The listing builds one solid part. Answer for the finished solid, in the listing's coordinates (mm). A direction names the side the tool comes from. Coordinates: 2 decimals unless noted, no trailing zeros. Order: outer loops, then holes, each group sorted by start corner. A loop starts at its lowest first (then second) coordinate and runs counter-clockwise, first axis right, second up. Notation, with made-up numbers: (65.25, -10) -> (88.25, -10) arc R22 ccw to (88.25, 24) -> close; hole circle Ø8 at (-3.75, 62.5). An arc over 180 degrees is marked (long way). Return JSON: item names as keys, results as strings.
```python
from build123d import *

# Parameters (mm, degrees)
SKETCH1_R                        = 9
BOSS_EXTRUDE1_DEPTH              = 40
M24_TAPPED_HOLE1_D               = 21
FILLET1_R                        = 10
SKETCH3_R                        = 9
SKETCH3_R_2                      = 9.680977079
BOSS_EXTRUDE2_DEPTH              = 25
M14_TAPPED_HOLE1_D               = 12
M14_TAPPED_HOLE1_DEPTH           = 40
M14_TAPPED_HOLE1_ON_FACE_2_D     = 12
M14_TAPPED_HOLE1_ON_FACE_2_DEPTH = 40


with BuildPart() as part:
    # Sketch1 → Boss-Extrude1 (new body)
    with BuildSketch(Plane.XY):
        Polygon((0, 215), (1520, 215), (1520, 120), (1420, 120), (1420, 0), (0, 0), align=None)
        with Locations((400, 166)):
            Circle(SKETCH1_R, mode=Mode.SUBTRACT)
        with Locations((280, 131)):
            Circle(SKETCH1_R, mode=Mode.SUBTRACT)
        with Locations((660, 131)):
            Circle(SKETCH1_R, mode=Mode.SUBTRACT)
        with Locations((1000, 166)):
            Circle(SKETCH1_R, mode=Mode.SUBTRACT)
    extrude(amount=BOSS_EXTRUDE1_DEPTH)

    # M24 Tapped Hole1 (through all)
    with Locations(Plane(origin=(780, 75, 40), x_dir=(1, 0, 0), z_dir=(0, 0, 1))):
        with Locations((0, 0), (-580, 0)):
            Hole(M24_TAPPED_HOLE1_D / 2)

    # Fillet1
    fillet1_edges = [part.edges().sort_by_distance(p)[0] for p in [
        (1520, 215, 20),
        (1520, 120, 20),
        (1420, 120, 20),
    ]]
    fillet(fillet1_edges, radius=FILLET1_R)

    # Sketch3 → Boss-Extrude2 (add)
    with BuildSketch(Plane(origin=(0, 0, 0), x_dir=(-1, 0, 0), z_dir=(0, 0, -1))):
        with Locations(Location((-1000, 166, 0), (0, 0, 90))):
            Circle(SKETCH3_R)
        with Locations((-400, 166)):
            Circle(SKETCH3_R_2)
    extrude(amount=-BOSS_EXTRUDE2_DEPTH)

    # M14 Tapped Hole1
    with Locations(Plane(origin=(1000, 166, 40), x_dir=(0, 1, 0), z_dir=(0, 0, 1))):
        with Locations((0, 0)):
            Hole(M14_TAPPED_HOLE1_D / 2, depth=M14_TAPPED_HOLE1_DEPTH)

    # M14 Tapped Hole1 on face 2
    with Locations(Plane(origin=(400, 166, 25), x_dir=(1, 0, 0), z_dir=(0, 0, 1))):
        with Locations((0, 0)):
            Hole(M14_TAPPED_HOLE1_ON_FACE_2_D / 2, depth=M14_TAPPED_HOLE1_ON_FACE_2_DEPTH)


solid = part.part
```
Item 1: Find the intervals of material crossed by probe 1 along X at (y, z) = (129.5, 27.5); probe 2 along X at (y, z) = (72.5, 5); probe 3 along Y at (x, z) = (400, 9), in increasing order.
Answer list:
{"probe 1": "0 to 271.13, 288.87 to 651.13, 668.87 to 1519.99", "probe 2": "0 to 189.8, 210.2 to 769.8, 790.2 to 1420", "probe 3": "0 to 160, 172 to 215"}
Item 2: The part is cut by section A-A on z = 17.5. Determine the outline of the cut face in (x, y), plus the area to 3 significant figures.
Answer list:
{"outline": "(0, 0) -> (1420, 0) -> (1420, 110) arc R10 cw to (1430, 120) -> (1510, 120) arc R10 ccw to (1520, 130) -> (1520, 205) arc R10 ccw to (1510, 215) -> (0, 215) -> close; hole circle Ø21 at (200, 75); hole circle Ø18 at (280, 131); hole circle Ø12 at (400, 166); hole circle Ø18 at (660, 131); hole circle Ø21 at (780, 75); hole circle Ø12 at (1000, 166)", "area": "313,000 mm2"}
Item 3: The part is cut by section B-B on y = 36.5. Determine the outline of the cut face in (x, z).
Answer list:
{"outline": "(0, 0) -> (1420, 0) -> (1420, 40) -> (0, 40) -> close"}
Item 4: A flat-ended cylindrical pin translates along its axis: pin 1 (20 mm diameter, centred on y = 75.5, z = 28.5, fed in from +X). Find the tip coordinate at first contact, or state that the pin passes through.
Answer list:
{"pin 1": "x = 1420"}
Item 5: Which of the six approach directions +Z, -Z, +X, -X, +Y, -Y give full straight-line access (tool end or side, diameter ignored) to faces 1 (the flat face through (1420, 56, 20)), 2 (the flat face through (744, 215, 20))?
Answer list:
{"face 1": "+Z, -Z, +X, -Y", "face 2": "+Z, -Z, +X, -X, +Y"}
